Here's how the part is built. I have some questions about the finished solid (model axes, mm). Face numbers are marked on the shaded views. A direction names the side the tool comes from. Round coordinates to 2 decimals unless told otherwise and drop trailing zeros. Loops run counter-clockwise (first coordinate to the right, second up) from the corner with the lowest first, then second, coordinate; pieces in that order, holes last. Notation, with made-up numbers: M 4,89 L 8,89 A7 ccw 8,97 Z; hole C 42.25,50.25 d11. An arc over 180 degrees is marked long. Use a Markdown table: item, result.
```python
from build123d import *

# Parameters (mm, degrees)
BASE_LIP_SKETCH_22_R       = 11
BASE_LIP_22_DEPTH          = 1
GROOVE_SKETCH_19_R         = 9.5
GROOVE_NECK_19_DEPTH       = 1
SHANK_SKETCH_22_R          = 11
SHANK_22_DEPTH             = 12
COLLAR_SKETCH_24_R         = 12
COLLAR_24_DEPTH            = 1
FLANGE_LOWER_SKETCH_35_R   = 17.5
FLANGE_LOWER_STEP_35_DEPTH = 1.5
FLANGE_SKETCH_36_R         = 18
FLANGE_36_DEPTH            = 1.5
SIDE_WINDOW_CUT_DEPTH      = 3
BOLT_HOLES_SKETCH_8X_3_R   = 1.5
BOLT_HOLES_8X_3_DEPTH      = 6
RECESS_SKETCH_14_R         = 7
RECESS_14_DEPTH            = 4
INNER_SPIGOT_SKETCH_10_R   = 5
INNER_SPIGOT_10_DEPTH      = 4
BORE_SKETCH_6_R            = 3
THROUGH_BORE_6_DEPTH       = 10.58


with BuildPart() as part:
    # Base Lip Sketch Ø22 → Base Lip Ø22 (new body)
    with BuildSketch(Plane(origin=(0, 0, 0), x_dir=(1, 0, 0), z_dir=(0, 1, 0))):
        with Locations(Location((0, 0, 0), (0, 0, 270))):
            Circle(BASE_LIP_SKETCH_22_R)
    extrude(amount=BASE_LIP_22_DEPTH)

    # Groove Sketch Ø19 → Groove Neck Ø19 (add)
    with BuildSketch(Plane(origin=(0, 1, 0), x_dir=(1, 0, 0), z_dir=(0, 1, 0))):
        with Locations(Location((0, 0, 0), (0, 0, 270))):
            Circle(GROOVE_SKETCH_19_R)
    extrude(amount=GROOVE_NECK_19_DEPTH)

    # Shank Sketch Ø22 → Shank Ø22 (add)
    with BuildSketch(Plane(origin=(0, 2, 0), x_dir=(1, 0, 0), z_dir=(0, 1, 0))):
        with Locations(Location((0, 0, 0), (0, 0, 270))):
            Circle(SHANK_SKETCH_22_R)
    extrude(amount=SHANK_22_DEPTH)

    # Collar Sketch Ø24 → Collar Ø24 (add)
    with BuildSketch(Plane(origin=(0, 14, 0), x_dir=(1, 0, 0), z_dir=(0, 1, 0))):
        with Locations(Location((0, 0, 0), (0, 0, 270))):
            Circle(COLLAR_SKETCH_24_R)
    extrude(amount=COLLAR_24_DEPTH)

    # Flange Lower Sketch Ø35 → Flange Lower Step Ø35 (add)
    with BuildSketch(Plane(origin=(0, 15, 0), x_dir=(1, 0, 0), z_dir=(0, 1, 0))):
        with Locations(Location((0, 0, 0), (0, 0, 270))):
            Circle(FLANGE_LOWER_SKETCH_35_R)
    extrude(amount=FLANGE_LOWER_STEP_35_DEPTH)

    # Flange Sketch Ø36 → Flange Ø36 (add)
    with BuildSketch(Plane(origin=(0, 16.5, 0), x_dir=(1, 0, 0), z_dir=(0, 1, 0))):
        with Locations(Location((0, 0, 0), (0, 0, 270))):
            Circle(FLANGE_SKETCH_36_R)
    extrude(amount=FLANGE_36_DEPTH)

    # Side Window Sketch → Side Window Cut (cut, symmetric)
    with BuildSketch(Plane.XY):
        with BuildLine():
            Line((-8, 0), (8, 0))
            ThreePointArc((8, 0), (6.634312477, 4.474361508), (3, 7.42))
            Line((3, 7.42), (-3, 7.42))
            ThreePointArc((-3, 7.42), (-6.634312477, 4.474361508), (-8, 0))
        make_face()
    extrude(amount=SIDE_WINDOW_CUT_DEPTH, both=True, mode=Mode.SUBTRACT)

    # Bolt Holes Sketch 8xØ3 → Bolt Holes 8xØ3 (cut)
    with BuildSketch(Plane(origin=(0, 18, 0), x_dir=(1, 0, 0), z_dir=(0, 1, 0))):
        with Locations(Location((0, 15, 0), (0, 0, 270))):
            Circle(BOLT_HOLES_SKETCH_8X_3_R)
        with Locations(Location((10.606601718, 10.606601718, 0), (0, 0, 270))):
            Circle(BOLT_HOLES_SKETCH_8X_3_R)
        with Locations(Location((15, 0, 0), (0, 0, 270))):
            Circle(BOLT_HOLES_SKETCH_8X_3_R)
        with Locations(Location((10.606601718, -10.606601718, 0), (0, 0, 270))):
            Circle(BOLT_HOLES_SKETCH_8X_3_R)
        with Locations(Location((0, -15, 0), (0, 0, 270))):
            Circle(BOLT_HOLES_SKETCH_8X_3_R)
        with Locations(Location((-10.606601718, -10.606601718, 0), (0, 0, 270))):
            Circle(BOLT_HOLES_SKETCH_8X_3_R)
        with Locations(Location((-15, 0, 0), (0, 0, 270))):
            Circle(BOLT_HOLES_SKETCH_8X_3_R)
        with Locations(Location((-10.606601718, 10.606601718, 0), (0, 0, 270))):
            Circle(BOLT_HOLES_SKETCH_8X_3_R)
    extrude(amount=-BOLT_HOLES_8X_3_DEPTH, mode=Mode.SUBTRACT)

    # Recess Sketch Ø14 → Recess Ø14 (cut)
    with BuildSketch(Plane(origin=(0, 18, 0), x_dir=(1, 0, 0), z_dir=(0, 1, 0))):
        with Locations(Location((0, 0, 0), (0, 0, 270))):
            Circle(RECESS_SKETCH_14_R)
    extrude(amount=-RECESS_14_DEPTH, mode=Mode.SUBTRACT)

    # Inner Spigot Sketch Ø10 → Inner Spigot Ø10 (add)
    with BuildSketch(Plane(origin=(0, 18, 0), x_dir=(1, 0, 0), z_dir=(0, 1, 0))):
        with Locations(Location((0, 0, 0), (0, 0, 270))):
            Circle(INNER_SPIGOT_SKETCH_10_R)
    extrude(amount=-INNER_SPIGOT_10_DEPTH)

    # Bore Sketch Ø6 → Through Bore Ø6 (cut)
    with BuildSketch(Plane(origin=(0, 18, 0), x_dir=(1, 0, 0), z_dir=(0, 1, 0))):
        with Locations(Location((0, 0, 0), (0, 0, 270))):
            Circle(BORE_SKETCH_6_R)
    extrude(amount=-THROUGH_BORE_6_DEPTH, mode=Mode.SUBTRACT)


solid = part.part
```
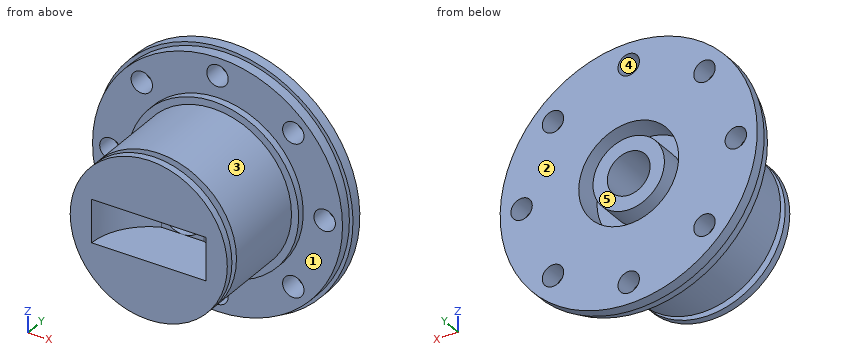
Q1. Imagine slicing it at D-D, the plane x = -10. Please give me the cut outline in (y, z), then the cut area to 3 significant figures.
Return value:
| item | result |
|---|---|
| outline | M 0,-4.58 L 1,-4.58 L 1,4.58 L 0,4.58 Z; M 2,-4.58 L 14,-4.58 L 14,-6.63 L 15,-6.63 L 15,-9.23 L 18,-9.23 L 18,9.23 L 15,9.23 L 15,6.63 L 14,6.63 L 14,4.58 L 2,4.58 Z; M 15,-14.36 L 16.5,-14.36 L 16.5,-14.97 L 18,-14.97 L 18,-11.98 L 15,-11.98 Z; M 15,11.98 L 18,11.98 L 18,14.97 L 16.5,14.97 L 16.5,14.36 L 15,14.36 Z |
| area | 204 mm^2 |
Q2. Imagine slicing it at C-C, the plane z = -13. Please give me the cut outline in (x, y), then the cut area to 3 significant figures.
Return value:
| item | result |
|---|---|
| outline | M -12.45,16.5 L -11.72,16.5 L -11.72,15 L 11.72,15 L 11.72,16.5 L 12.45,16.5 L 12.45,18 L -12.45,18 Z |
| area | 72.5 mm^2 |
Q3. I need wall thicknesses on line 1 (X direction, y = 16.05, z = 0); line 2 (X direction, y = 14.25, z = 0); line 3 (Y direction, x = 7.5, z = -6). Which ranges of each line are inside material? Lowest first, please. Write a range as from..to.
Return value:
| item | result |
|---|---|
| line 1 | x = -17.5..-16.5, -13.5..-7, -5..-3, 3..5, 7..13.5, 16.5..17.5 |
| line 2 | x = -12..-7, -5..-3, 3..5, 7..12 |
| line 3 | y = 0..1, 2..18 |
Q4. Imagine slicing it at B-B, the plane x = -15. Please give me the cut outline in (y, z), then the cut area to 3 significant figures.
Return value:
| item | result |
|---|---|
| outline | M 15,-9.01 L 16.5,-9.01 L 16.5,-9.95 L 18,-9.95 L 18,-1.5 L 15,-1.5 Z; M 15,1.5 L 18,1.5 L 18,9.95 L 16.5,9.95 L 16.5,9.01 L 15,9.01 Z |
| area | 47.9 mm^2 |
Q5. Imagine slicing it at A-A, the plane y = 12.75. Please give me the cut outline in (x, z), then the cut area to 3 significant figures.
Return value:
| item | result |
|---|---|
| outline | C 0,0 d22; hole C 0,0 d6 |
| area | 352 mm^2 |
Q6. Will these pins go through, and if not, where does the flat tip stop? P1, Ø5, axis at x = 0, z = 15, coming from the -Y side; P2, Ø5, axis at y = 9.5, z = 1.5, coming from the +X side; P3, Ø2, axis at x = 3.5, y = 15, coming from the +Z side; P4, Ø1.8, axis at x = 15, z = 0, coming from the -Y side (1 decimal).
Return value:
| item | result |
|---|---|
| P1 | stops at y = 15 |
| P2 | stops at x = 11 |
| P3 | stops at z = 17.32 |
| P4 | passes through |
Q7. We'd pull the mould along Z, two halves only. Please class the marked faces 3, 4 and 5: pulls with the +Z half, pulls with the -Z half, needs draft (parallel to the pull), parting line crosses it, or undercut.
Return value:
| item | result |
|---|---|
| face 3 | parting line crosses it |
| face 4 | undercut |
| face 5 | needs draft |
Q8. For the marked faces 1 and 2, which set-ups out of +Z, -Z, +X, -X, +Y, -Y let a thin tool reach every point of the face, with its end or its side?
Return value:
| item | result |
|---|---|
| face 1 | -Y |
| face 2 | +Z, -Z, +X, -X, +Y |
